```python
from build123d import *

# Parameters (mm, degrees)
SKETCH1_W               = 10
SKETCH1_H               = 18
BOSS_EXTRUDE1_DEPTH     = 6
SKETCH2_R               = 1.75
CUT_EXTRUDE1_DEPTH      = 10
CHAMFER1_SIZE           = 1
M2_5_TAPPED_HOLE1_D     = 2.05
M2_5_TAPPED_HOLE1_DEPTH = 6.35
M2_5_TAPPED_HOLE1_TIP   = 0.615882135


with BuildPart() as part:
    # Sketch1 → Boss-Extrude1 (new body)
    with BuildSketch(Plane(origin=(0, 0, 0), x_dir=(1, 0, 0), z_dir=(0, 1, 0))):
        Rectangle(SKETCH1_W, SKETCH1_H)
    extrude(amount=BOSS_EXTRUDE1_DEPTH)

    # Sketch2 → Cut-Extrude1 (cut)
    with BuildSketch(Plane(origin=(0, 6, 0), x_dir=(1, 0, 0), z_dir=(0, 1, 0))):
        with Locations(Location((1.5, 5, 0), (0, 0, 270))):
            Circle(SKETCH2_R)
        with Locations(Location((1.5, -5, 0), (0, 0, 270))):
            Circle(SKETCH2_R)
    extrude(amount=-CUT_EXTRUDE1_DEPTH, mode=Mode.SUBTRACT)

    # Chamfer1
    chamfer1_edges = [part.edges().sort_by_distance(p)[0] for p in [
        (5, 3, 9),
        (5, 3, -9),
    ]]
    chamfer(chamfer1_edges, length=CHAMFER1_SIZE)

    # M2.5 Tapped Hole1
    with Locations(Plane(origin=(-5, 3, -6), x_dir=(0, 0, -1), z_dir=(-1, 0, 0))):
        with Locations((0, 0), (-12, 0)):
            Hole(M2_5_TAPPED_HOLE1_D / 2, depth=M2_5_TAPPED_HOLE1_DEPTH)
            with Locations((0, 0, -(M2_5_TAPPED_HOLE1_DEPTH + M2_5_TAPPED_HOLE1_TIP / 2))):  # 118° drill point
                Cone(0, M2_5_TAPPED_HOLE1_D / 2, M2_5_TAPPED_HOLE1_TIP, mode=Mode.SUBTRACT)


solid = part.part
```
Read the model definition and answer for the solid it produces. Units are mm, in the model's axes. A direction names the side the tool comes from. Give positions to 0.01 mm unless a question says otherwise; leave off trailing zeros. Order: outer loops, then holes, each group sorted by start corner. A loop starts at its lowest first (then second) coordinate and runs counter-clockwise, first axis right, second up.
(1) Find section B-B (y = 1). Give the vertices of the cut face in (x, z), plus the area to 3 significant figures.
(2) For faces 4 (the flat face through (-1, 3, 9)), 5 (the cylindrical face through (-2.486, 2.955, -7.024)), determine the directions among +Z, -Z, +X, -X, +Y, -Y from which every point of the face is accessible in a straight line to the end or side of a thin tool.
(3) Find section A-A (z = -6). Give the vertices of the cut face in (x, y) (3 decimals).
(4) Find section C-C (z = -3.5). Give the vertices of the cut face in (x, y), plus the area to 3 significant figures.
(5) Find section D-D (x = -3.5). Give the vertices of the cut face in (y, z) (3 decimals).
(6) Straight lines are drawn through the part: L1, parallel to X at y = 4, z = -5; L2, parallel to Y at x = -1.5, z = 6 (3 decimals); L3, parallel to Z at x = -2.5, y = 2.75. For each, find the intervals that lie inside material, in ascending order.
(7) For a pull along X with two mould halves and no side action, classify faces 1 (the cylindrical face through (3, 3, -4.1)), 2 (the flat face through (0, 6, 0)), 3 (the flat face through (4.5, 3, -8.5)) as released by +X, released by -X, zero draft, split by the parting line, or undercut.
Result sheet:
1. outline: (-5, -9) - (4, -9) - (5, -8) - (5, 8) - (4, 9) - (-5, 9) - close; hole circle Ø3.5 at (1.5, -5); hole circle Ø3.5 at (1.5, 5)
1. area: 160 mm2
2. face 4: +Z, +X, -X, +Y, -Y
2. face 5: -X
3. outline: (-5, 0) - (0.064, 0) - (0.064, 1.975) - (-5, 1.975) - close; (-5, 4.025) - (0.064, 4.025) - (0.064, 6) - (-5, 6) - close; (2.936, 0) - (5, 0) - (5, 6) - (2.936, 6) - close
4. outline: (-5, 0) - (0.6, 0) - (0.6, 6) - (-5, 6) - close; (2.4, 0) - (5, 0) - (5, 6) - (2.4, 6) - close
4. area: 49.2 mm2
5. outline: (0, -9) - (6, -9) - (6, 9) - (0, 9) - close; hole circle Ø2.05 at (3, -6); hole circle Ø2.05 at (3, 6)
6. L1: x = -5 to -0.25, 3.25 to 5
6. L2: y = 0 to 1.975, 4.025 to 6
6. L3: z = -9 to -6.99, -5.01 to 5.01, 6.99 to 9
7. face 1: undercut
7. face 2: zero draft
7. face 3: released by +X
